from build123d import *

# Parameters (mm, degrees)
CUT_EXTRUDE1_DEPTH = 4


with BuildPart() as part:
    # Sketch1 → Revolve1 (revolve)
    with BuildSketch(Plane.XY, mode=Mode.PRIVATE) as revolve1_sk:
        Polygon((-13, 0), (-13, 3.233), (-12.233, 4), (-3.767, 4), (-3.0905, 3.3235), (-1, 3.3235), (-1, 5), (0, 5), (0, 8.5), (19, 10), (39, 10), (39, 0), align=None)
    revolve(revolve1_sk.sketch.rotate(Axis((39, 0, 0), (-1, 0, 0)), 270), axis=Axis((39, 0, 0), (-1, 0, 0)))

    # Sketch2 → Cut-Extrude1 (cut)
    with BuildSketch(Plane(origin=(-13, 0, 0), x_dir=(0, 0, -1), z_dir=(1, 0, 0))):
        Polygon((-2, 1.154700538), (-2, -1.154700538), (0, -2.309401077), (2, -1.154700538), (2, 1.154700538), (0, 2.309401077), align=None)
    extrude(amount=CUT_EXTRUDE1_DEPTH, mode=Mode.SUBTRACT)

    # Sketch3 → Cut-Revolve1 (revolve, cut)
    with BuildSketch(Plane.XY, mode=Mode.PRIVATE) as cut_revolve1_sk:
        Polygon((-9, 0), (-9, 2.309401077), (-7.67, 0), align=None)
    revolve(cut_revolve1_sk.sketch.rotate(Axis((-7.67, 0, 0), (-1, 0, 0)), 270), axis=Axis((-7.67, 0, 0), (-1, 0, 0)), mode=Mode.SUBTRACT)


solid = part.part
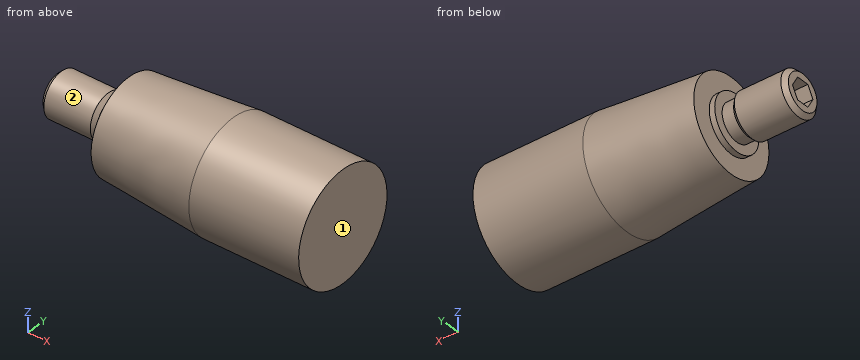
For this review, take the finished solid that the model builds, in its own axes (mm). Face numbers are marked on the shaded views. A direction names the side the tool comes from. Round coordinates to 2 decimals unless told otherwise and drop trailing zeros. Loops run counter-clockwise (first coordinate to the right, second up) from the corner with the lowest first, then second, coordinate; pieces in that order, holes last. Notation, with made-up numbers: (24, 13) - (45, 13) arc R21 ccw to (45, 22) - close; hole circle Ø1 at (61.5, 48). An arc over 180 degrees is marked (long way). Use one line per item in the form item = value.
Item 1: Clearance check with flat-ended pins moving along their axes: P1, Ø10, axis at x = 8.5, z = -3.5, coming from the +Y side; P2, Ø1, axis at y = -6.5, z = 4.5, coming from the -X side; P3, Ø2.5, axis at x = -12, y = 0.5, coming from the +Z side; P4, Ø5, axis at x = 25.5, y = 2.5, coming from the -Z side. State where each tip first meets the part, or that it passes through.
Answers:
P1 = 9.47
P2 = 0
P3 = 4
P4 = -10
Item 2: Consider section B-B on x = -5.5. Write out the cut boundary in (y, z), then the cut area to 3 significant figures.
Answers:
outline = circle Ø8 at (0, 0)
area = 50.3 mm^2
Item 3: Consider section A-A on x = 24.5. Write out the cut boundary in (y, z), then the cut area to 3 significant figures.
Answers:
outline = circle Ø20 at (0, 0)
area = 314 mm^2
Item 4: For line 1 (X direction, y = 0.75, z = 4.25); line 2 (X direction, y = 2, z = 6.5); line 3 (Z direction, x = 2, y = -1), list the stretches that pass through material, from the lowest coordinate up.
Answers:
line_1 = -1 to 39
line_2 = 0 to 39
line_3 = -8.6 to 8.6
Item 5: Tool access review of the marked faces 1 and 2: name each direction out of +Z, -Z, +X, -X, +Y, -Y from which nothing blocks a thin tool from reaching the whole face with its end or side.
Answers:
face_1 = +Z, -Z, +X, +Y, -Y
face_2 = -X
